Read the model definition and answer for the solid it produces. Units are mm, in the model's axes. Face numbers are marked on the shaded views. A direction names the side the tool comes from. Coordinates: 2 decimals unless noted, no trailing zeros. Write each loop counter-clockwise with the first axis right and the second up, starting at its lowest first coordinate (ties: lowest second). Pieces come first, ordered by that corner, then holes. Notation, with made-up numbers: M 79.5,45 L 130.5,45 A20 ccw 130.5,59 Z; hole C 70,36.25 d2. An arc over 180 degrees is marked long. Write item = value, one per line.
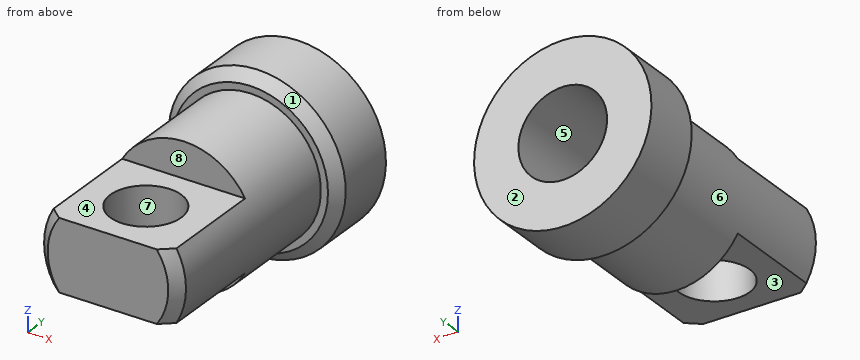
from build123d import *

# Parameters (mm, degrees)
SKETCH1_R             = 2
BOSS_EXTRUDE1_DEPTH   = 6
SKETCH2_R             = 2.5
BOSS_EXTRUDE2_DEPTH   = 2
M3_TAPPED_HOLE1_D     = 2.5
M3_TAPPED_HOLE1_DEPTH = 4.5
M3_TAPPED_HOLE1_TIP   = 0.751075774
CHAMFER1_SIZE         = 0.3
SKETCH6_R             = 1
CUT_EXTRUDE1_DEPTH    = 5
SKETCH7_W             = 3
SKETCH7_H             = 3.2
CUT_EXTRUDE2_DEPTH    = 5


with BuildPart() as part:
    # Sketch1 → Boss-Extrude1 (new body)
    with BuildSketch(Plane(origin=(0, 0, 0), x_dir=(1, 0, 0), z_dir=(0, 1, 0))):
        with Locations(Location((0, 0, 0), (0, 0, 270))):
            Circle(SKETCH1_R)
    extrude(amount=BOSS_EXTRUDE1_DEPTH)

    # Sketch2 → Boss-Extrude2 (add)
    with BuildSketch(Plane(origin=(0, 6, 0), x_dir=(1, 0, 0), z_dir=(0, 1, 0))):
        with Locations(Location((0, 0, 0), (0, 0, 270))):
            Circle(SKETCH2_R)
    extrude(amount=BOSS_EXTRUDE2_DEPTH)

    # M3 Tapped Hole1
    with Locations(Plane(origin=(0, 8, 0), x_dir=(1, 0, 0), z_dir=(0, 1, 0))):
        with Locations((0, 0)):
            Hole(M3_TAPPED_HOLE1_D / 2, depth=M3_TAPPED_HOLE1_DEPTH)
            with Locations((0, 0, -(M3_TAPPED_HOLE1_DEPTH + M3_TAPPED_HOLE1_TIP / 2))):  # 118° drill point
                Cone(0, M3_TAPPED_HOLE1_D / 2, M3_TAPPED_HOLE1_TIP, mode=Mode.SUBTRACT)

    # Chamfer1
    chamfer1_edges = [part.edges().sort_by_distance(p)[0] for p in [
        (0, 0, -2),
        (0, 6, -2.5),
    ]]
    chamfer(chamfer1_edges, length=CHAMFER1_SIZE)

    # Sketch6 → Cut-Extrude1 (cut, symmetric)
    with BuildSketch(Plane.XY):
        with Locations(Location((0, 1.6, 0), (0, 0, 90.00000001))):
            Circle(SKETCH6_R)
    extrude(amount=CUT_EXTRUDE1_DEPTH, both=True, mode=Mode.SUBTRACT)

    # Sketch7 → Cut-Extrude2 (cut, symmetric)
    with BuildSketch(Plane(origin=(0, 0, 0), x_dir=(0, 0, -1), z_dir=(1, 0, 0))):
        with Locations((2.5, 1.6)):
            Rectangle(SKETCH7_W, SKETCH7_H)
        with Locations((-2.5, 1.6)):
            Rectangle(SKETCH7_W, SKETCH7_H)
    extrude(amount=CUT_EXTRUDE2_DEPTH, both=True, mode=Mode.SUBTRACT)


solid = part.part
Item 1: Consider line 1 along Z through (x, y) = (0, 5.35); line 2 along X through (y, z) = (6.25, 1.05); line 3 along X through (y, z) = (7.5, -1.8). Determine where each line is inside the solid, lowest interval first. Write a range as from..to.
Worked answers:
line_1 = -2..-1.25, 1.25..2
line_2 = -2.21..-0.68, 0.68..2.21
line_3 = -1.73..1.73
Item 2: Flat-ended cylindrical pins translate along their axes: pin 1 (1.6 mm diameter, centred on x = -1, y = 2, fed in from +Z); pin 2 (0.8 mm diameter, centred on x = 0.5, z = 1.5, fed in from -Y); pin 3 (3 mm diameter, centred on x = 0, y = 1.6, fed in from -Z). Find the tip coordinate at first contact, or state that the pin passes through.
Worked answers:
pin_1 = 1
pin_2 = 3.2
pin_3 = -1
Item 3: For a pull along Y with two mould halves and no side action, classify the marked faces 6, 7 and 8 as released by +Y, released by -Y, zero draft, split by the parting line, or undercut.
Worked answers:
face_6 = zero draft
face_7 = undercut
face_8 = released by -Y
Item 4: Find section B-B (y = 6.5). Determine the outline of the cut face in (x, z).
Worked answers:
outline = C 0,0 d5; hole C 0,0 d2.5
Item 5: Which of the six approach directions +Z, -Z, +X, -X, +Y, -Y give full straight-line access (tool end or side, diameter ignored) to the marked faces 1, 2, 3, 4 and 5?
Worked answers:
face_1 = -Y
face_2 = +Z, -Z, +X, -X, +Y
face_3 = -Z, +X, -X, -Y
face_4 = +Z, +X, -X, -Y
face_5 = +Y
Item 6: Find section A-A (y = 1.6). Determine the outline of the cut face in (x, z), and give its area (3 significant figures).
Worked answers:
outline = M -1.73,-1 L -1,-1 L -1,1 L -1.73,1 A2 ccw Z; M 1,-1 L 1.73,-1 A2 ccw 1.73,1 L 1,1 Z
area = 3.65 mm²
